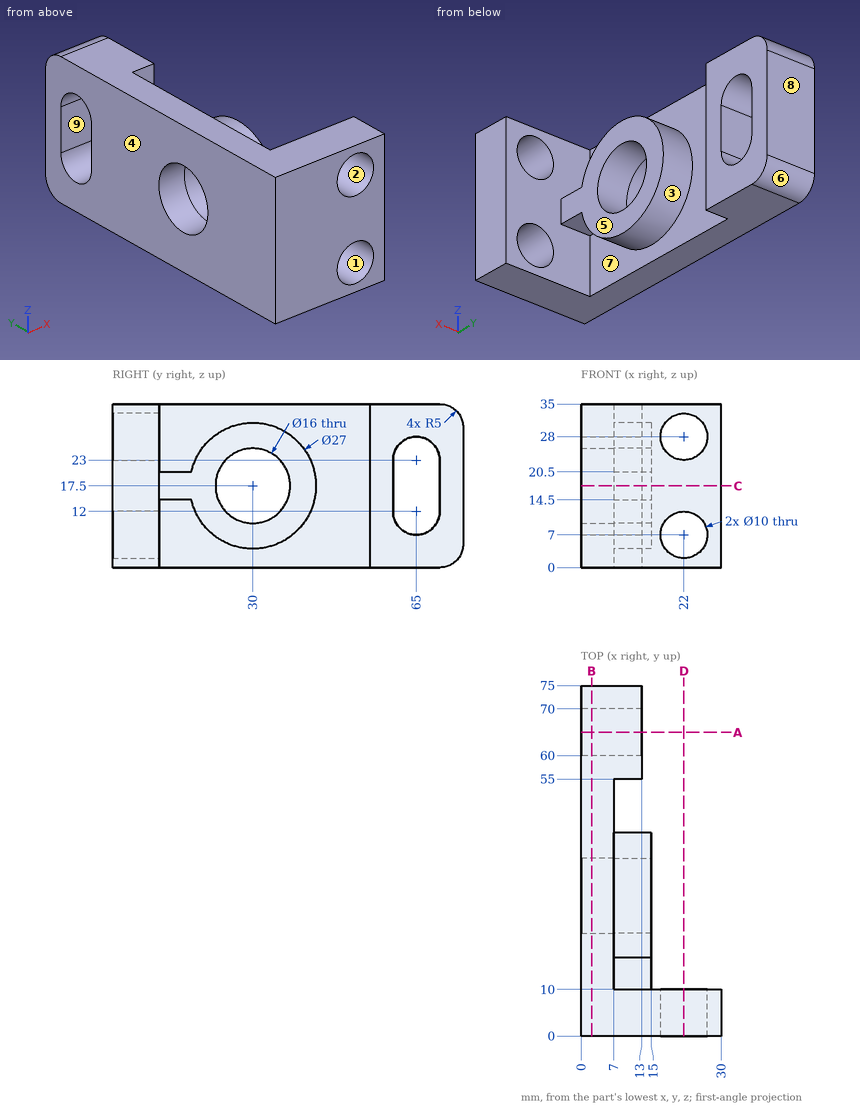
Can you work these out from the drawing? Everything is in mm from the part's minimum corner. A direction names the side the tool comes from. Coordinates: 2 decimals unless noted, no trailing zeros. Loops run counter-clockwise (first coordinate to the right, second up) from the corner with the lowest first, then second, coordinate; pieces in that order, holes last. Notation, with made-up numbers: (-23.5, 48) - (13.5, 48) arc R22 ccw to (13.5, 85) - close; hole circle Ø5 at (-26, 82). An arc over 180 degrees is marked (long way). Put each result on its own line as item: value. Start each with the question number.
Item 1: For pin 1 (6 mm diameter, centred on x = 16.5, y = 25.5, fed in from +Z); pin 2 (9 mm diameter, centred on x = 22, z = 7, fed in from -Y); pin 3 (21 mm diameter, centred on y = 30, z = 17.5, fed in from +X), each with a flat end and sliding along its axis, tell me the tip position at first contact or that it passes through.
Item 2: If I drill on line 1 along X through (y, z) = (7, 7); line 2 along Y through (x, z) = (10.75, 27.5); line 3 along X through (y, z) = (14.5, 5), over which ranges is the centre line in solid material (lowest first)?
Item 3: If we mould it in two halves opening along X, with no side actions, what happens to the marked faces 1, 2, 3 and 4? For each: +X half, -X half, draft (parallel to the pull), parting line (faces both ways), or undercut.
Item 4: Suppose I cut it at A-A (y = 65). Please give me the cut outline in (x, z).
Item 5: Suppose I cut it at C-C (z = 17.5). Please give me the cut outline in (x, y), and give its area (3 significant figures).
Item 6: Which directions (+Z, -Z, +X, -X, +Y, -Y) give clear straight access to the entire face, cutting with the end or side of a thin tool? Please do the marked faces 5, 6, 7, 8 and 9.
Item 7: Suppose I cut it at D-D (x = 22). Please give me the cut outline in (y, z).
Item 8: Suppose I cut it at B-B (x = 2.25). Please give me the cut outline in (y, z).
Here are the results:
1. pin 1: z = 30.87
1. pin 2: through
1. pin 3: x = 15
2. line 1: 0 to 17, 27 to 30
2. line 2: 0 to 10, 20.93 to 39.07, 55 to 62.82, 67.18 to 75
2. line 3: 0 to 7
3. face 1: undercut
3. face 2: undercut
3. face 3: draft
3. face 4: -X half
4. outline: (0, 0) - (13, 0) - (13, 7) - (0, 7) - close; (0, 28) - (13, 28) - (13, 35) - (0, 35) - close
5. outline: (0, 0) - (30, 0) - (30, 10) - (15, 10) - (15, 22) - (0, 22) - close; (0, 38) - (15, 38) - (15, 43.5) - (7, 43.5) - (7, 55) - (13, 55) - (13, 60) - (0, 60) - close; (0, 70) - (13, 70) - (13, 75) - (0, 75) - close
5. area: 773 mm²
6. face 5: +Z, -Z, +X, +Y
6. face 6: -Z, +X, -X, +Y
6. face 7: +X
6. face 8: +Z, -Z, +X, -X, +Y
6. face 9: +X, -X
7. outline: (0, 0) - (10, 0) - (10, 2) - (0, 2) - close; (0, 12) - (10, 12) - (10, 23) - (0, 23) - close; (0, 33) - (10, 33) - (10, 35) - (0, 35) - close
8. outline: (0, 0) - (70, 0) arc R5 ccw to (75, 5) - (75, 30) arc R5 ccw to (70, 35) - (0, 35) - close; hole circle Ø16 at (30, 17.5); hole (60, 12) arc R5 ccw to (70, 12) - (70, 23) arc R5 ccw to (60, 23) - close
